from build123d import *

# Parameters (mm, degrees)
SKETCH1_R           = 16
BOSS_EXTRUDE1_DEPTH = 14


with BuildPart() as part:
    # Sketch1 → Boss-Extrude1 (new body)
    with BuildSketch(Plane.XY):
        Polygon((0, 0), (40, 0), (200, -160), (200, -200), (40, -200), (0, -160), align=None)
        with Locations((88, -112)):
            Circle(SKETCH1_R, mode=Mode.SUBTRACT)
    extrude(amount=BOSS_EXTRUDE1_DEPTH)


solid = part.part
CAD build for the part. Positions are in the model's coordinates, mm. Coordinates: 2 decimals unless noted, no trailing zeros. Order: outer loops, then holes, each group sorted by start corner. A loop starts at its lowest first (then second) coordinate and runs counter-clockwise, first axis right, second up. Notation, with made-up numbers: (-37.5, -30.75) -> (7.5, -30.75) arc R25 cw to (7.5, 4.25) -> close; hole circle Ø5 at (52.5, -5). An arc over 180 degrees is marked (long way). Answer in a Markdown table with one row per item.
1) Drill centre lines: line 1 (Y direction, x = 88, z = 6.75); line 2 (X direction, y = -104, z = 3.5); line 3 (X direction, y = -117.5, z = 8.5). Where is each one in solid material? Low to high.
Check values:
| item | result |
|---|---|
| line 1 | -200 to -128, -96 to -48 |
| line 2 | 0 to 74.14, 101.86 to 144 |
| line 3 | 0 to 72.98, 103.02 to 157.5 |
2) Band-saw the part on C-C (z = 3.5). List the corners of the cut face in (x, y), and give its area (3 significant figures).
Check values:
| item | result |
|---|---|
| outline | (0, -160) -> (40, -200) -> (200, -200) -> (200, -160) -> (40, 0) -> (0, 0) -> close; hole circle Ø32 at (88, -112) |
| area | 25,600 mm2 |
3) Flat gauge pins, fed straight in: P1, Ø5, axis at x = 57.5, z = 11.5, coming from the +Y side; P2, Ø5, axis at x = 65, z = 7, coming from the +Y side. Where does each tip first touch, or does it go through?
Check values:
| item | result |
|---|---|
| P1 | y = -15 |
| P2 | y = -22.5 |
4) Band-saw the part on A-A (y = -112). List the corners of the cut face in (x, z).
Check values:
| item | result |
|---|---|
| outline | (0, 0) -> (72, 0) -> (72, 14) -> (0, 14) -> close; (104, 0) -> (152, 0) -> (152, 14) -> (104, 14) -> close |
5) Mould opens along Y. For faces 1 (the face through (200, -180, 7)), 2 (the face through (76.207, -101.186, 6.902)), 3 (the face through (20, -180, 7)), 4 (the face through (20, 0, 7)) say: pulls with the +Y half, pulls with the -Y half, needs draft (parallel to the pull), parting line crosses it, or undercut.
Check values:
| item | result |
|---|---|
| face 1 | needs draft |
| face 2 | undercut |
| face 3 | pulls with the -Y half |
| face 4 | pulls with the +Y half |
6) Band-saw the part on B-B (x = 88). List the corners of the cut face in (y, z).
Check values:
| item | result |
|---|---|
| outline | (-200, 0) -> (-128, 0) -> (-128, 14) -> (-200, 14) -> close; (-96, 0) -> (-48, 0) -> (-48, 14) -> (-96, 14) -> close |
7) Band-saw the part on D-D (x = 45). List the corners of the cut face in (y, z).
Check values:
| item | result |
|---|---|
| outline | (-200, 0) -> (-5, 0) -> (-5, 14) -> (-200, 14) -> close |
